Verification items for the finished model (mm, model axes). Give positions to 0.01 mm unless a question says otherwise; leave off trailing zeros. Loops run counter-clockwise (first coordinate to the right, second up) from the corner with the lowest first, then second, coordinate; pieces in that order, holes last. Notation, with made-up numbers: (74, 9) - (126, 9) arc R21 cw to (126, 33) - close; hole circle Ø5 at (74.5, -15.75). An arc over 180 degrees is marked (long way). Use one line per item in the form item = value.
```python
from build123d import *

# Parameters (mm, degrees)
SKETCH_1_W          = 3.85
SKETCH_1_H          = 51
EXTRUDE_1_DEPTH     = 80
CUT_EXTRUDE_1_REACH = 1465.749
SKETCH_2_R          = 2.1


with BuildPart() as part:
    # 草图1 → 凸台-拉伸1 (new body)
    with BuildSketch(Plane.XY):
        with Locations((-0.405329913, -17.044468303)):
            Rectangle(SKETCH_1_W, SKETCH_1_H)
    extrude(amount=EXTRUDE_1_DEPTH)

    # 草图2 → 切除-拉伸1 (cut, up to next)
    with BuildSketch(Plane(origin=(5.369670087, -1051.794731348, 1009.143932915), x_dir=(0, -1, 0), z_dir=(1, 0, 0)), mode=Mode.PRIVATE) as cut_extrude_1_sk1:
        with Locations((-1055.250263055, 981.942263912)):
            Circle(SKETCH_2_R)
    cut_extrude_1_tool1 = extrude(cut_extrude_1_sk1.sketch, amount=-CUT_EXTRUDE_1_REACH, mode=Mode.PRIVATE) & part.part
    # 草图2 → 切除-拉伸1 (cut, up to next)
    with BuildSketch(Plane(origin=(5.369670087, -1051.794731348, 1009.143932915), x_dir=(0, -1, 0), z_dir=(1, 0, 0)), mode=Mode.PRIVATE) as cut_extrude_1_sk2:
        with Locations((-1055.250263055, 958.292263912)):
            Circle(SKETCH_2_R)
    cut_extrude_1_tool2 = extrude(cut_extrude_1_sk2.sketch, amount=-CUT_EXTRUDE_1_REACH, mode=Mode.PRIVATE) & part.part
    # 草图2 → 切除-拉伸1 (cut, up to next)
    with BuildSketch(Plane(origin=(5.369670087, -1051.794731348, 1009.143932915), x_dir=(0, -1, 0), z_dir=(1, 0, 0)), mode=Mode.PRIVATE) as cut_extrude_1_sk3:
        with Locations((-1014.250263055, 958.292263912)):
            Circle(SKETCH_2_R)
    cut_extrude_1_tool3 = extrude(cut_extrude_1_sk3.sketch, amount=-CUT_EXTRUDE_1_REACH, mode=Mode.PRIVATE) & part.part
    # 草图2 → 切除-拉伸1 (cut, up to next)
    with BuildSketch(Plane(origin=(5.369670087, -1051.794731348, 1009.143932915), x_dir=(0, -1, 0), z_dir=(1, 0, 0)), mode=Mode.PRIVATE) as cut_extrude_1_sk4:
        with Locations((-1014.250263055, 981.942263912)):
            Circle(SKETCH_2_R)
    cut_extrude_1_tool4 = extrude(cut_extrude_1_sk4.sketch, amount=-CUT_EXTRUDE_1_REACH, mode=Mode.PRIVATE) & part.part
    add(cut_extrude_1_tool1.solids().sort_by_distance((5.36967, 3.455532, 27.201669))[0], mode=Mode.SUBTRACT)
    add(cut_extrude_1_tool2.solids().sort_by_distance((5.36967, 3.455532, 50.851669))[0], mode=Mode.SUBTRACT)
    add(cut_extrude_1_tool3.solids().sort_by_distance((5.36967, -37.544468, 50.851669))[0], mode=Mode.SUBTRACT)
    add(cut_extrude_1_tool4.solids().sort_by_distance((5.36967, -37.544468, 27.201669))[0], mode=Mode.SUBTRACT)


solid = part.part
```
1. Draft check along Z on faces 1 (the cylindrical face through (-0.38, 2.33, 25.43)), 2 (the flat face through (0, -17, 80)), 3 (the flat face through (1.52, -17, 39)). Enter one of: released by +Z, released by -Z, zero draft, split by the parting line, or undercut.
Result set:
face_1 = undercut
face_2 = released by +Z
face_3 = zero draft
2. Scan lines: probe 1 along Y at (x, z) = (0.15, 49); probe 2 along Z at (x, y) = (1.15, -36); probe 3 along Z at (x, y) = (-0.9, 4). Record each from-to range of solid material in increasing order.
Result set:
probe_1 = -42.54 to -38.54, -36.55 to 2.46, 4.45 to 8.46
probe_2 = 0 to 25.78, 28.62 to 49.43, 52.27 to 80
probe_3 = 0 to 25.17, 29.23 to 48.82, 52.88 to 80
3. Section check A-A, the plane y = -38. Record the cut outline in (x, z).
Result set:
outline = (-2.33, 0) - (1.52, 0) - (1.52, 25.15) - (-2.33, 25.15) - close; (-2.33, 29.25) - (1.52, 29.25) - (1.52, 48.8) - (-2.33, 48.8) - close; (-2.33, 52.9) - (1.52, 52.9) - (1.52, 80) - (-2.33, 80) - close
